Read the model definition and answer for the solid it produces. Units are mm, in the model's axes. A direction names the side the tool comes from. Round coordinates to 2 decimals unless told otherwise and drop trailing zeros. Write each loop counter-clockwise with the first axis right and the second up, starting at its lowest first coordinate (ties: lowest second). Pieces come first, ordered by that corner, then holes. Notation, with made-up numbers: (-19, 24.5) -> (11, 24.5) arc R18 cw to (11, 45.5) -> close; hole circle Ø7 at (7.5, 6.25). An arc over 180 degrees is marked (long way). Return JSON: item names as keys, results as strings.
from build123d import *
from OCP.BRepFilletAPI import BRepFilletAPI_MakeChamfer

# Parameters (mm, degrees)
SKETCH1_R           = 6.5
BOSS_EXTRUDE1_DEPTH = 8
CUT_EXTRUDE1_DEPTH  = 4
SKETCH3_R           = 4
BOSS_EXTRUDE2_DEPTH = 55
CHAMFER1_SIZE       = 1
FILLET1_R           = 1
CHAMFER2_SIZE       = 1.729106628
CHAMFER2_SIZE2      = 2.994900532
FILLET2_R           = 0.1


with BuildPart() as part:
    # Sketch1 → Boss-Extrude1 (new body)
    with BuildSketch(Plane.XY):
        Circle(SKETCH1_R)
    extrude(amount=BOSS_EXTRUDE1_DEPTH)

    # Sketch2 → Cut-Extrude1 (cut)
    with BuildSketch(Plane.XY.offset(8)):
        Polygon((3, 1.732050808), (0, 3.464101615), (-3, 1.732050808), (-3, -1.732050808), (0, -3.464101615), (3, -1.732050808), align=None)
    extrude(amount=-CUT_EXTRUDE1_DEPTH, mode=Mode.SUBTRACT)

    # Sketch3 → Boss-Extrude2 (add)
    with BuildSketch(Plane(origin=(0, 0, 0), x_dir=(-1, 0, 0), z_dir=(0, 0, -1))):
        with Locations(Location((0, 0, 0), (0, 0, 180))):
            Circle(SKETCH3_R)
    extrude(amount=BOSS_EXTRUDE2_DEPTH)

    # Chamfer1
    chamfer1_edges = [part.edges().sort_by_distance(p)[0] for p in [
        (-4, 0, -55),
    ]]
    chamfer(chamfer1_edges, length=CHAMFER1_SIZE)

    # Fillet1
    fillet1_edges = [part.edges().sort_by_distance(p)[0] for p in [
        (-6.5, 0, 8),
    ]]
    fillet(fillet1_edges, radius=FILLET1_R)

    # Chamfer2: one chamfer whose edges measure the first distance from different faces: ONE call of the kernel's chamfer builder (chamfer() names one face for all edges)
    chamfer2_edges_1 = [part.edges().sort_by_distance(p)[0] for p in [
        (-1.5, 2.598076211, 4),
    ]]
    chamfer2_side_1 = [part.faces().sort_by_distance(p)[0] for p in [
        (-1.5, 2.598076211, 6),
    ]]
    chamfer2_edges_2 = [part.edges().sort_by_distance(p)[0] for p in [
        (1.5, 2.598076211, 4),
    ]]
    chamfer2_side_2 = [part.faces().sort_by_distance(p)[0] for p in [
        (1.5, 2.598076211, 6),
    ]]
    chamfer2_edges_3 = [part.edges().sort_by_distance(p)[0] for p in [
        (3, 0, 4),
    ]]
    chamfer2_side_3 = [part.faces().sort_by_distance(p)[0] for p in [
        (3, 0, 6),
    ]]
    chamfer2_edges_4 = [part.edges().sort_by_distance(p)[0] for p in [
        (1.5, -2.598076211, 4),
    ]]
    chamfer2_side_4 = [part.faces().sort_by_distance(p)[0] for p in [
        (1.5, -2.598076211, 6),
    ]]
    chamfer2_edges_5 = [part.edges().sort_by_distance(p)[0] for p in [
        (-1.5, -2.598076211, 4),
    ]]
    chamfer2_side_5 = [part.faces().sort_by_distance(p)[0] for p in [
        (-1.5, -2.598076211, 6),
    ]]
    chamfer2_edges_6 = [part.edges().sort_by_distance(p)[0] for p in [
        (-3, 0, 4),
    ]]
    chamfer2_side_6 = [part.faces().sort_by_distance(p)[0] for p in [
        (-3, 0, 6),
    ]]
    chamfer2 = BRepFilletAPI_MakeChamfer(part.part.solid().wrapped)
    for e in chamfer2_edges_1:
        chamfer2.Add(CHAMFER2_SIZE, CHAMFER2_SIZE2, e.wrapped, chamfer2_side_1[0].wrapped)  # the first distance lies on this face
    for e in chamfer2_edges_2:
        chamfer2.Add(CHAMFER2_SIZE, CHAMFER2_SIZE2, e.wrapped, chamfer2_side_2[0].wrapped)  # the first distance lies on this face
    for e in chamfer2_edges_3:
        chamfer2.Add(CHAMFER2_SIZE, CHAMFER2_SIZE2, e.wrapped, chamfer2_side_3[0].wrapped)  # the first distance lies on this face
    for e in chamfer2_edges_4:
        chamfer2.Add(CHAMFER2_SIZE, CHAMFER2_SIZE2, e.wrapped, chamfer2_side_4[0].wrapped)  # the first distance lies on this face
    for e in chamfer2_edges_5:
        chamfer2.Add(CHAMFER2_SIZE, CHAMFER2_SIZE2, e.wrapped, chamfer2_side_5[0].wrapped)  # the first distance lies on this face
    for e in chamfer2_edges_6:
        chamfer2.Add(CHAMFER2_SIZE, CHAMFER2_SIZE2, e.wrapped, chamfer2_side_6[0].wrapped)  # the first distance lies on this face
    add(Compound.cast(chamfer2.Shape()), mode=Mode.REPLACE)

    # Fillet2
    fillet2_edges = [part.edges().sort_by_distance(p)[0] for p in [
        (-4, 0, 0),
    ]]
    fillet(fillet2_edges, radius=FILLET2_R)


solid = part.part
Item 1: Section B-B (z = -43) is taken. Give the vertices of the cut face in (x, y).
Worked answers:
{"outline": "circle Ø8 at (0, 0)"}
Item 2: Flat-ended cylindrical pins translate along their axes: pin 1 (0.7 mm diameter, centred on y = -1, z = 7, fed in from +X); pin 2 (6 mm diameter, centred on x = 4, z = -10, fed in from +Y); pin 3 (1.5 mm diameter, centred on x = 0.5, z = -38.5, fed in from -Y); pin 4 (1 mm diameter, centred on x = 5, z = -8.5, fed in from -Y). Find the tip coordinate at first contact, or state that the pin passes through.
Worked answers:
{"pin 1": "stops at x = 6.47", "pin 2": "stops at y = 3.87", "pin 3": "stops at y = -4", "pin 4": "passes through"}
Item 3: Section A-A (z = 3) is taken. Give the vertices of the cut face in (x, y).
Worked answers:
{"outline": "circle Ø13 at (0, 0)"}
Item 4: A tool of negligible diameter and unlimited length cuts with its end or side. For faces 1 (the flat face through (1.4, -4.2, 0)), 2 (the flat face through (3, 0, 7)), 3 (the flat face through (0, 0, -55)), from which of +Z, -Z, +X, -X, +Y, -Y can it reach the whole face along a straight path? Write none if from no direction.
Worked answers:
{"face 1": "-Z", "face 2": "+Z", "face 3": "-Z, +X, -X, +Y, -Y"}
Item 5: For a pull along X with two mould halves and no side action, classify faces 4 (the cylindrical face through (-5.158, -3.955, 3.451)), 5 (the flat face through (2.4, -2.4, 8)), 6 (the flat face through (1.81, -0.02, 5.04)) as released by +X, released by -X, zero draft, split by the parting line, or undercut.
Worked answers:
{"face 4": "split by the parting line", "face 5": "zero draft", "face 6": "undercut"}
Item 6: Straight lines are drawn through the part: L1, parallel to Z at x = 1, y = -4.25; L2, parallel to Y at x = -2, z = -10; L3, parallel to X at y = -0.25, z = -45.5. For each, find the intervals that lie inside material, in ascending order. Write a range as [from, to].
Worked answers:
{"L1": "z = [0, 8]", "L2": "y = [-3.46, 3.46]", "L3": "x = [-3.99, 3.99]"}
